Verification items for the finished model (mm, model axes). Give positions to 0.01 mm unless a question says otherwise; leave off trailing zeros. Loops run counter-clockwise (first coordinate to the right, second up) from the corner with the lowest first, then second, coordinate; pieces in that order, holes last. Notation, with made-up numbers: M 67.25,81 L 86.25,81 A28 ccw 86.25,108 Z; hole C 53,-26.5 d6. An arc over 180 degrees is marked long. Use CSV: the item, a comma, the result in double quotes.
from build123d import *

# Parameters (mm, degrees)
EXTRUDE_1_DEPTH = 19


with BuildPart() as part:
    # 草图2 → 拉伸-薄壁1 (new, symmetric)
    with BuildSketch(Plane.XY):
        with BuildLine():
            Line((250.396106976, 303.41117138), (93.71226198, -42.453604657))
            ThreePointArc((93.71226198, -42.453604657), (0, -102.880025838), (-93.71226198, -42.453604657))
            Line((-93.71226198, -42.453604657), (-250.396106976, 303.41117138))
            ThreePointArc((-250.396106976, 303.41117138), (-255.847210975, 311.746098094), (-263.566345627, 318.03899078))
            Line((-263.566345627, 318.03899078), (-542.021364981, 481.241496264))
            ThreePointArc((-542.021364981, 481.241496264), (-589.286880464, 596.951990053), (-490, 672.88))
            Line((-490, 672.88), (490, 672.88))
            ThreePointArc((490, 672.88), (589.286880464, 596.951990053), (542.021364981, 481.241496264))
            Line((542.021364981, 481.241496264), (263.566345627, 318.03899078))
            ThreePointArc((263.566345627, 318.03899078), (255.847210975, 311.746098094), (250.396106976, 303.41117138))
        make_face()
        with BuildLine():
            Line((245.841661895, 305.474428516), (89.1578169, -40.390347521))
            ThreePointArc((89.1578169, -40.390347521), (0, -97.880025838), (-89.1578169, -40.390347521))
            Line((-89.1578169, -40.390347521), (-245.841661895, 305.474428516))
            ThreePointArc((-245.841661895, 305.474428516), (-252.131397279, 315.091651647), (-261.038091108, 322.352681669))
            Line((-261.038091108, 322.352681669), (-539.493110463, 485.555187153))
            ThreePointArc((-539.493110463, 485.555187153), (-584.461507191, 595.642114953), (-490, 667.88))
            Line((-490, 667.88), (490, 667.88))
            ThreePointArc((490, 667.88), (584.461507191, 595.642114953), (539.493110463, 485.555187153))
            Line((539.493110463, 485.555187153), (261.038091108, 322.352681669))
            ThreePointArc((261.038091108, 322.352681669), (252.131397279, 315.091651647), (245.841661895, 305.474428516))
        make_face(mode=Mode.SUBTRACT)
    extrude(amount=EXTRUDE_1_DEPTH, both=True)


solid = part.part
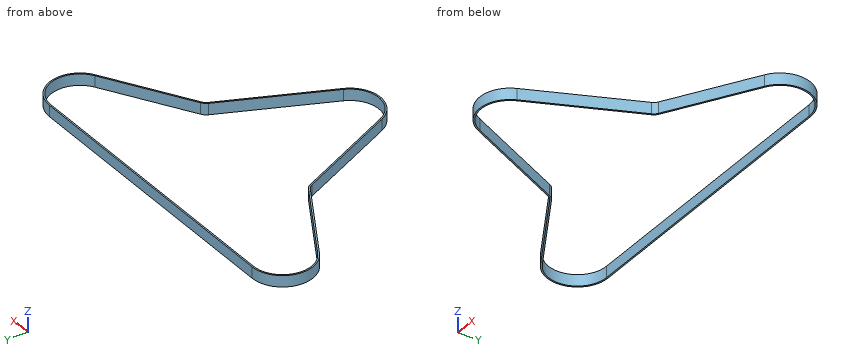
(1) Section check A-A on z = 0.5. Record the cut outline in (x, y), plus the area to 3 significant figures.
Calculated:
outline,"M -542.02,481.24 L -263.57,318.04 A32.5 cw -250.4,303.41 L -93.71,-42.45 A102.88 ccw 93.71,-42.45 L 250.4,303.41 A32.5 cw 263.57,318.04 L 542.02,481.24 A102.88 ccw 490,672.88 L -490,672.88 A102.88 ccw Z; hole M -539.49,485.56 L -261.04,322.35 A37.5 cw -245.84,305.47 L -89.16,-40.39 A97.88 ccw 89.16,-40.39 L 245.84,305.47 A37.5 cw 261.04,322.35 L 539.49,485.56 A97.88 ccw 490,667.88 L -490,667.88 A97.88 ccw Z"
area,"15,900 mm²"
(2) Section check B-B on x = -511. Record the cut outline in (y, z), plus the area to 3 significant figures.
Calculated:
outline,"M 463.06,-19 L 468.86,-19 L 468.86,19 L 463.06,19 Z; M 665.6,-19 L 670.71,-19 L 670.71,19 L 665.6,19 Z"
area,"415 mm²"
(3) Scan lines: L1, parallel to Y at x = 376, z = -6; L2, parallel to Y at x = -379.5, z = -11; L3, parallel to X at y = 618.5, z = 13. Record each from-to range of solid material in increasing order. Write a range as from..to.
Calculated:
L1,"y = 383.94..389.73, 667.88..672.88"
L2,"y = 385.99..391.78, 667.88..672.88"
L3,"x = -580.73..-575.02, 575.02..580.73"
(4) Section check C-C on y = 405.5. Record the cut outline in (x, z), plus the area to 3 significant figures.
Calculated:
outline,"M -412.79,-19 L -402.9,-19 L -402.9,19 L -412.79,19 Z; M 402.9,-19 L 412.79,-19 L 412.79,19 L 402.9,19 Z"
area,"752 mm²"
(5) Depth check by flat-ended pin: pin 1 Ø19 at (x, z) = (-27.5, -4.5) entering from -Y; pin 2 Ø4 at (y, z) = (10, -2) entering from +X; pin 3 Ø3 at (y, z) = (560, 2) entering from -X. Enter the tip coordinate at first touch or a pass-through.
Calculated:
pin 1,"stops at y = -101.29"
pin 2,"stops at x = 118.38"
pin 3,"stops at x = -592.53"
